Could you check a few things on this model? Use its own coordinates, in mm. A direction names the side the tool comes from. Coordinates: 2 decimals unless noted, no trailing zeros. Order: outer loops, then holes, each group sorted by start corner. A loop starts at its lowest first (then second) coordinate and runs counter-clockwise, first axis right, second up. Notation, with made-up numbers: (11.5, 87) - (35.5, 87) arc R16 cw to (35.5, 105) - close; hole circle Ø6 at (-30, 35.5). An arc over 180 degrees is marked (long way). Answer as a JSON object with one key per item and string values. Group by question number.
(1) Imagine slicing it at C-C, the plane x = 0. Write out the boundary of the cut face in (y, z), and give its area (3 significant figures).
(2) We'd pull the mould along Z, two halves only. Please class faces 6 (the cylindrical face through (41.99, 7.47, 9.92)), 7 (the flat face through (-1, 5, 24)), 8 (the flat face through (-1, 10, -11)): pulls with the +Z half, pulls with the -Z half, needs draft (parallel to the pull), parting line crosses it, or undercut.
(3) Will these pins go through, and if not, where does the flat tip stop? P1, Ø2, axis at y = 4, z = -0.5, coming from the -X side; P2, Ø10.5, axis at x = 38, z = 12, coming from the -Y side; P3, Ø4.5, axis at x = -3.5, z = -0.5, coming from the +Y side.
(4) Imagine slicing it at B-B, the plane z = 12. Write out the boundary of the cut face in (x, y) (3 decimals).
(5) Imagine slicing it at D-D, the plane z = 0. Write out the boundary of the cut face in (x, y), and give its area (4 significant figures).
(6) Which directions (+Z, -Z, +X, -X, +Y, -Y) give clear straight access to the entire face, cutting with the end or side of a thin tool? Please do faces 1 (the flat face through (-70, 5, 10)), 2 (the flat face through (-75, 5, -17)), 3 (the flat face through (70, 5, 10)), 4 (the cylindrical face through (41.99, 7.47, -14.08)), 5 (the cylindrical face through (45.32, 2.48, 13.63)).
(7) Imagine slicing it at A-A, the plane y = 8. Write out the boundary of the cut face in (x, z), and give its area (3 significant figures).
(8) Please list where these lines run through material, in increasing order: probe 1 along Z at (x, y) = (-38, 2.5); probe 2 along X at (y, z) = (8.1, 12); probe 3 along Z at (x, y) = (-38, 8.05).
from build123d import *

# Parameters (mm, degrees)
SKETCH1_W                                  = 150
SKETCH1_H                                  = 48
BOSS_EXTRUDE1_DEPTH                        = 10
CBORE_FOR_M8_CHEESE_HEAD_SCREW1_AT_2_COUNT = 2
CBORE_FOR_M8_CHEESE_HEAD_SCREW1_AT_2_PITCH = 76
CBORE_FOR_M8_CHEESE_HEAD_SCREW1_AT_3_COUNT = 2
CBORE_FOR_M8_CHEESE_HEAD_SCREW1_AT_3_PITCH = 24
CBORE_FOR_M8_CHEESE_HEAD_SCREW1_AT_4_COUNT = 2
CBORE_FOR_M8_CHEESE_HEAD_SCREW1_AT_4_PITCH = 79.699435381
SKETCH6_R                                  = 7.5
CUT_EXTRUDE2_DEPTH                         = 5
SKETCH7_W                                  = 20
SKETCH7_H                                  = 20
CUT_EXTRUDE3_DEPTH                         = 80.37883849


with BuildPart() as part:
    # Sketch1 → Boss-Extrude1 (new body)
    with BuildSketch(Plane(origin=(0, 0, 0), x_dir=(1, 0, 0), z_dir=(0, 1, 0))):
        Rectangle(SKETCH1_W, SKETCH1_H)
    extrude(amount=BOSS_EXTRUDE1_DEPTH)

    # Sketch4 → CBORE for M8 Cheese Head Screw1 (revolve, cut)
    with BuildSketch(Plane(origin=(38, 0, 12), x_dir=(0, 0, -1), z_dir=(1, 0, 0))):
        Polygon((0, 0), (0, 12.703872786), (4.5, 10), (4.5, 5), (7.5, 5), (7.5, 0.025), (7.525, 0), align=None)
    cbore_for_m8_cheese_head_screw1 = revolve(axis=Axis((38, -6.35, 12), (0, 1, 0)), mode=Mode.SUBTRACT)

    # CBORE for M8 Cheese Head Screw1 at 2: CBORE for M8 Cheese Head Screw1 ×2
    with Locations(*[(-i * CBORE_FOR_M8_CHEESE_HEAD_SCREW1_AT_2_PITCH, 0, 0) for i in range(1, CBORE_FOR_M8_CHEESE_HEAD_SCREW1_AT_2_COUNT)]):
        add(cbore_for_m8_cheese_head_screw1, mode=Mode.SUBTRACT)

    # CBORE for M8 Cheese Head Screw1 at 3: CBORE for M8 Cheese Head Screw1 ×2
    with Locations(*[(0, 0, -i * CBORE_FOR_M8_CHEESE_HEAD_SCREW1_AT_3_PITCH) for i in range(1, CBORE_FOR_M8_CHEESE_HEAD_SCREW1_AT_3_COUNT)]):
        add(cbore_for_m8_cheese_head_screw1, mode=Mode.SUBTRACT)

    # CBORE for M8 Cheese Head Screw1 at 4: CBORE for M8 Cheese Head Screw1 ×2
    with Locations(*[Vector(-0.9535826651341417, 0, -0.3011313679370974) * (i * CBORE_FOR_M8_CHEESE_HEAD_SCREW1_AT_4_PITCH) for i in range(1, CBORE_FOR_M8_CHEESE_HEAD_SCREW1_AT_4_COUNT)]):
        add(cbore_for_m8_cheese_head_screw1, mode=Mode.SUBTRACT)

    # Sketch6 → Cut-Extrude2 (cut)
    with BuildSketch(Plane(origin=(0, 10, 0), x_dir=(1, 0, 0), z_dir=(0, 1, 0))):
        with Locations(Location((0, 0, 0), (0, 0, 270))):
            Circle(SKETCH6_R)
    extrude(amount=-CUT_EXTRUDE2_DEPTH, mode=Mode.SUBTRACT)

    # Sketch7 → Cut-Extrude3 (cut, through all)
    with BuildSketch(Plane(origin=(0, 10, 0), x_dir=(1, 0, 0), z_dir=(0, 1, 0))):
        with Locations((75, 0)):
            Rectangle(SKETCH7_W, SKETCH7_H)
        with Locations((-75, 0)):
            Rectangle(SKETCH7_W, SKETCH7_H)
    extrude(amount=-CUT_EXTRUDE3_DEPTH, mode=Mode.SUBTRACT)


solid = part.part
Result set:
{
 "1": {"outline": "(0, -24) - (10, -24) - (10, -7.5) - (5, -7.5) - (5, 7.5) - (10, 7.5) - (10, 24) - (0, 24) - close", "area": "405 mm^2"},
 "2": {"face 6": "undercut", "face 7": "pulls with the +Z half", "face 8": "needs draft"},
 "3": {"P1": "stops at x = -65", "P2": "stops at y = 5", "P3": "stops at y = 5"},
 "4": {"outline": "(-75, 0) - (-45.525, 0) - (-45.5, 0.025) - (-45.5, 5) - (-42.5, 5) - (-42.5, 10) - (-75, 10) - close; (-33.5, 5) - (-30.5, 5) - (-30.5, 0.025) - (-30.475, 0) - (30.475, 0) - (30.5, 0.025) - (30.5, 5) - (33.5, 5) - (33.5, 10) - (-33.5, 10) - close; (42.5, 5) - (45.5, 5) - (45.5, 0.025) - (45.525, 0) - (75, 0) - (75, 10) - (42.5, 10) - close"},
 "5": {"outline": "(-65, 0) - (65, 0) - (65, 10) - (7.5, 10) - (7.5, 5) - (-7.5, 5) - (-7.5, 10) - (-65, 10) - close", "area": "1,225 mm^2"},
 "6": {"face 1": "-X, +Y, -Y", "face 2": "+Z, -Z, -X, +Y, -Y", "face 3": "+X, +Y, -Y", "face 4": "+Y, -Y", "face 5": "-Y"},
 "7": {"outline": "(-75, -24) - (75, -24) - (75, -10) - (65, -10) - (65, 10) - (75, 10) - (75, 24) - (-75, 24) - (-75, 10) - (-65, 10) - (-65, -10) - (-75, -10) - close; hole circle Ø9 at (-38, -12); hole circle Ø9 at (-38, 12); hole circle Ø15 at (0, 0); hole circle Ø9 at (38, -12); hole circle Ø9 at (38, 12)", "area": "6,370 mm^2"},
 "8": {"probe 1": "z = -24 to -19.5, -4.5 to 4.5, 19.5 to 24", "probe 2": "x = -75 to -42.5, -33.5 to 33.5, 42.5 to 75", "probe 3": "z = -24 to -16.5, -7.5 to 7.5, 16.5 to 24"}
}
